Geometry: see drawing. Coordinates: mm, zero at the bounding-box minimum. Give positions to 0.01 mm unless a question says otherwise; leave off trailing zeros. Order: outer loops, then holes, each group sorted by start corner. A loop starts at its lowest first (then second) coordinate and runs counter-clockwise, first axis right, second up. Notation, with made-up numbers: M 39,10 L 57,10 A30 cw 57,37 Z; hole C 11,-22 d3. An arc over 180 degrees is marked long. Write item = value, one per line. Start each with the question number.
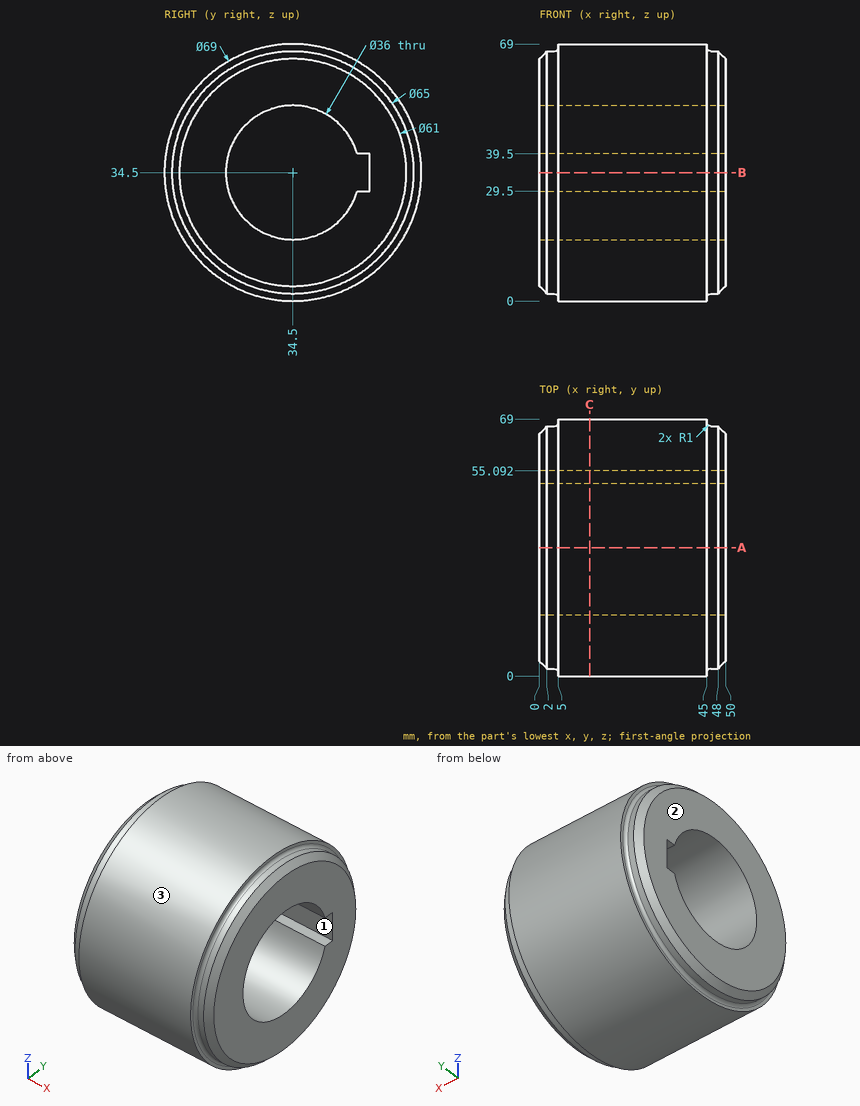
1) Cut plane A-A (y = 34.5). Return loops of the section in (x, z), plus the area to 3 significant figures.
2) Cut plane C-C (x = 13.5). Return loops of the section in (y, z).
3) Ray query, L1, parallel to Y at x = 34, z = 34.5; L2, parallel to Y at x = 35, z = 33; L3, parallel to Z at x = 37, y = 53. Return the intervals inside material, ascending.
4) Pin query (flat end, axial travel): pin 1 Ø1 at (x, z) = (25.5, 40) entering from +Y; pin 2 Ø1 at (x, y) = (19.5, 53) entering from -Z; pin 3 Ø10 at (x, z) = (14.5, 41.5) entering from +Y. Return the tip coordinate at first contact, or that it passes through.
5) Cut plane B-B (z = 34.5). Return loops of the section in (x, y), plus the area to 3 significant figures.
6) Draft query along Y for the marked faces 1, 2 and 3. Return one class per face: pulls with the +Y half, pulls with the -Y half, needs draft (parallel to the pull), parting line crosses it, or undercut.
Reply:
q1.outline = M 0,4 L 2,2 L 4,2 A1 cw 5,1 L 5,0 L 45,0 L 45,1 A1 cw 46,2 L 48,2 L 50,4 L 50,16.5 L 0,16.5 Z; M 0,52.5 L 50,52.5 L 50,65 L 48,67 L 46,67 A1 cw 45,68 L 45,69 L 5,69 L 5,68 A1 cw 4,67 L 2,67 L 0,65 Z
q1.area = 1,600 mm²
q2.outline = C 34.5,34.5 d69; hole M 51.79,29.5 L 55.09,29.5 L 55.09,39.5 L 51.79,39.5 A18 ccw long Z
q3.L1 = 0 to 16.5, 55.09 to 69
q3.L2 = 0.03 to 16.56, 55.09 to 68.97
q3.L3 = 5.38 to 29.5, 39.5 to 63.62
q4.pin_1 = 68.64
q4.pin_2 = 5.07
q4.pin_3 = 68.94
q5.outline = M 0,4 L 2,2 L 4,2 A1 cw 5,1 L 5,0 L 45,0 L 45,1 A1 cw 46,2 L 48,2 L 50,4 L 50,16.5 L 0,16.5 Z; M 0,55.09 L 50,55.09 L 50,65 L 48,67 L 46,67 A1 cw 45,68 L 45,69 L 5,69 L 5,68 A1 cw 4,67 L 2,67 L 0,65 Z
q5.area = 1,470 mm²
q6.face_1 = undercut
q6.face_2 = needs draft
q6.face_3 = parting line crosses it
